```python
from build123d import *

# Parameters (mm, degrees)
GB_6728_1986_080_X_40_X_4_1_DEPTH = 1089
HOLE_WIZARD_M6_1_D                = 5
SKETCH_4_R                        = 15
CUT_EXTRUDE_1_DEPTH               = 1091.468248048


with BuildPart() as part:
    # Sketch12 → Gb／6728-1986矩形空心型钢 080 X 40 X 4(1) (new body)
    with BuildSketch(Plane(origin=(0, 0, 0), x_dir=(0, 0, -1), z_dir=(1, 0, 0))):
        with BuildLine():
            Line((-12, -40), (12, -40))
            ThreePointArc((12, -40), (17.656854249, -37.656854249), (20, -32))
            Line((20, -32), (20, 32))
            ThreePointArc((20, 32), (17.656854249, 37.656854249), (12, 40))
            Line((12, 40), (-12, 40))
            ThreePointArc((-12, 40), (-17.656854249, 37.656854249), (-20, 32))
            Line((-20, 32), (-20, -32))
            ThreePointArc((-20, -32), (-17.656854249, -37.656854249), (-12, -40))
        make_face()
        with BuildLine():
            Line((-12, -36), (12, -36))
            ThreePointArc((12, -36), (14.828427125, -34.828427125), (16, -32))
            Line((16, -32), (16, 32))
            ThreePointArc((16, 32), (14.828427125, 34.828427125), (12, 36))
            Line((12, 36), (-12, 36))
            ThreePointArc((-12, 36), (-14.828427125, 34.828427125), (-16, 32))
            Line((-16, 32), (-16, -32))
            ThreePointArc((-16, -32), (-14.828427125, -34.828427125), (-12, -36))
        make_face(mode=Mode.SUBTRACT)
    extrude(amount=GB_6728_1986_080_X_40_X_4_1_DEPTH)

    # M6 螺纹孔1 (through all)
    with Locations(Plane(origin=(0, 0, -20), x_dir=(-1, 0, 0), z_dir=(0, 0, -1))):
        with Locations((-590, 0), (-750, 0), (-910, 0), (-1070, 0)):
            Hole(HOLE_WIZARD_M6_1_D / 2)

    # 草图4 → 切除-拉伸1 (cut, through all)
    with BuildSketch(Plane.XY.offset(20)):
        with Locations((1051, 0)):
            Circle(SKETCH_4_R)
    extrude(amount=-CUT_EXTRUDE_1_DEPTH, mode=Mode.SUBTRACT)


solid = part.part
```
For this review, take the finished solid that the model builds, in its own axes (mm). A direction names the side the tool comes from. Round coordinates to 2 decimals unless told otherwise and drop trailing zeros. Loops run counter-clockwise (first coordinate to the right, second up) from the corner with the lowest first, then second, coordinate; pieces in that order, holes last.
(1) Mouldability with a two-part tool opening along Y and no side actions: class faces 3 (the cylindrical face through (1065.307, 4.506, 18.028)), 4 (the flat face through (537, -40, 0)), 5 (the flat face through (537, 0, -20)), 6 (the flat face through (537, -36, 0)) as released by +Y, released by -Y, zero draft, split by the parting line, or undercut.
Returned:
face 3: undercut
face 4: released by -Y
face 5: zero draft
face 6: undercut
(2) Wall thickness on line 1 along Y through (x, z) = (981.5, 9); line 2 along Z through (x, y) = (212, -23); line 3 along Y through (x, z) = (1070, 19): over which ranges is each line inside the solid? List them lowest first.
Returned:
line 1: y = -40 to -36, 36 to 40
line 2: z = -20 to -16, 16 to 20
line 3: y = -35.87 to -2.5, 2.5 to 35.87
(3) Tool access review of faces 1 (the flat face through (537, 40, 0)), 2 (the flat face through (537, 0, -16)): name each direction out of +Z, -Z, +X, -X, +Y, -Y from which nothing blocks a thin tool from reaching the whole face with its end or side.
Returned:
face 1: +Z, -Z, +X, -X, +Y
face 2: +X, -X
(4) Clearance check with flat-ended pins moving along their axes: P1, Ø4, axis at x = 750, y = 0, coming from the +Z side; P2, Ø8, axis at x = 590, y = 0, coming from the +Z side. State where each tip first meets the part, or that it passes through.
Returned:
P1: passes through
P2: stops at z = 20
(5) We need section B-B (x = 1051). Give the boundary of the cut face in (y, z), plus the area to 3 significant figures.
Returned:
outline: (-40, -12) arc R8 ccw to (-32, -20) - (-15, -20) - (-15, -16) - (-32, -16) arc R4 cw to (-36, -12) - (-36, 12) arc R4 cw to (-32, 16) - (-15, 16) - (-15, 20) - (-32, 20) arc R8 ccw to (-40, 12) - close; (15, -20) - (32, -20) arc R8 ccw to (40, -12) - (40, 12) arc R8 ccw to (32, 20) - (15, 20) - (15, 16) - (32, 16) arc R4 cw to (36, 12) - (36, -12) arc R4 cw to (32, -16) - (15, -16) - close
area: 615 mm2
(6) We need section A-A (x = 463). Give the boundary of the cut face in (y, z).
Returned:
outline: (-40, -12) arc R8 ccw to (-32, -20) - (32, -20) arc R8 ccw to (40, -12) - (40, 12) arc R8 ccw to (32, 20) - (-32, 20) arc R8 ccw to (-40, 12) - close; hole (-36, -12) arc R4 ccw to (-32, -16) - (32, -16) arc R4 ccw to (36, -12) - (36, 12) arc R4 ccw to (32, 16) - (-32, 16) arc R4 ccw to (-36, 12) - close
